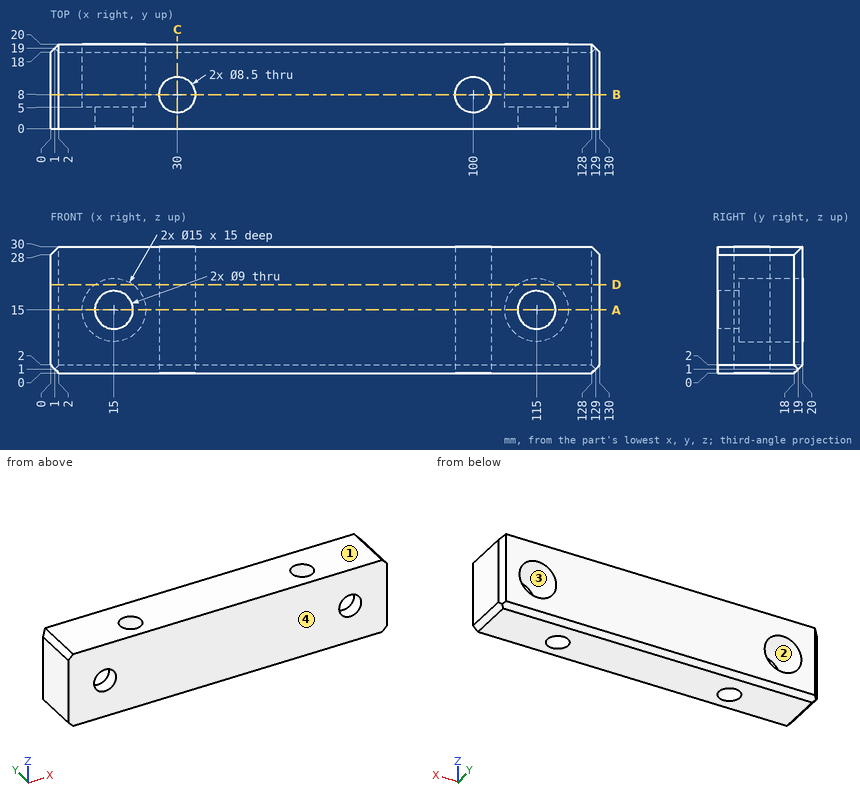
The figure shows three views and two pictorial views of one solid part (mm, origin at its lowest corner). Answer the questions. Give positions to 0.01 mm unless a question says otherwise; leave off trailing zeros. Loops run counter-clockwise (first coordinate to the right, second up) from the corner with the lowest first, then second, coordinate; pieces in that order, holes last. Notation, with made-up numbers: (-10, 78) - (39, 78) arc R19 cw to (39, 97) - close; hole circle Ø6 at (18.5, 50.25). An arc over 180 degrees is marked (long way). Use one line per item in the form item = value.
1. Section D-D on z = 21 is taken. Give the vertices of the cut face in (x, y).
Calculated:
outline = (0, 0) - (130, 0) - (130, 18) - (128, 20) - (119.5, 20) - (119.5, 5) - (110.5, 5) - (110.5, 20) - (19.5, 20) - (19.5, 5) - (10.5, 5) - (10.5, 20) - (2, 20) - (0, 18) - close; hole circle Ø8.5 at (30, 8); hole circle Ø8.5 at (100, 8)
2. Section A-A on z = 15 is taken. Give the vertices of the cut face in (x, y).
Calculated:
outline = (0, 0) - (10.5, 0) - (10.5, 5) - (7.5, 5) - (7.5, 20) - (2, 20) - (0, 18) - close; (19.5, 0) - (110.5, 0) - (110.5, 5) - (107.5, 5) - (107.5, 20) - (22.5, 20) - (22.5, 5) - (19.5, 5) - close; (119.5, 0) - (130, 0) - (130, 18) - (128, 20) - (122.5, 20) - (122.5, 5) - (119.5, 5) - close; hole circle Ø8.5 at (30, 8); hole circle Ø8.5 at (100, 8)
3. Section B-B on y = 8 is taken. Give the vertices of the cut face in (x, z), then the cut area to 3 significant figures.
Calculated:
outline = (0, 2) - (2, 0) - (25.75, 0) - (25.75, 30) - (2, 30) - (0, 28) - close; (34.25, 0) - (95.75, 0) - (95.75, 30) - (34.25, 30) - close; (104.25, 0) - (128, 0) - (130, 2) - (130, 28) - (128, 30) - (104.25, 30) - close; hole circle Ø15 at (15, 15); hole circle Ø15 at (115, 15)
area = 3,030 mm^2
4. The mould has two halves that part along Z. Classify the marked faces 1, 2, 3 and 4: pulls with the +Z half, pulls with the -Z half, needs draft (parallel to the pull), parting line crosses it, or undercut.
Calculated:
face_1 = pulls with the +Z half
face_2 = undercut
face_3 = undercut
face_4 = needs draft
5. Find the intervals of material crossed by line 1 along X through (y, z) = (6.5, 5); line 2 along Z through (x, y) = (15, 3.45); line 3 along Y through (x, z) = (100, 17.25), in increasing order. Write a range as [from, to].
Calculated:
line_1 = [0, 26.02], [33.98, 96.02], [103.98, 130]
line_2 = [0, 10.5], [19.5, 30]
line_3 = [0, 3.75], [12.25, 20]
6. Section C-C on x = 30 is taken. Give the vertices of the cut face in (y, z).
Calculated:
outline = (0, 0) - (3.75, 0) - (3.75, 30) - (0, 30) - close; (12.25, 0) - (18, 0) - (20, 2) - (20, 30) - (12.25, 30) - close
7. Given pin 1 Ø16.5 at (x, z) = (14, 18.5) entering from +Y; pin 2 Ø7.5 at (x, z) = (113, 14.5) entering from +Y, each flat-ended and moving along its own axis, determine where each tip first touches the part or whether it passes through.
Calculated:
pin_1 = 20
pin_2 = 5
